Could you check a few things on this model? Use its own coordinates, in mm. A direction names the side the tool comes from. Coordinates: 2 decimals unless noted, no trailing zeros. Loops run counter-clockwise (first coordinate to the right, second up) from the corner with the lowest first, then second, coordinate; pieces in that order, holes last. Notation, with made-up numbers: (8, 69) - (18, 69) arc R15 ccw to (18, 79) - close; hole circle Ø4 at (-32.75, 65.25). An arc over 180 degrees is marked (long way). One line per question, with ' | ' between items. Start each with the question number.
1. I want a section at C-C, the plane x = 0. Write out the boundary of the cut face in (y, z).
2. I'm going to push flat-ended pins straight in: P1, Ø1.5, axis at x = -8, y = 4, coming from the -Z side; P2, Ø3, axis at y = 1, z = 1.5, coming from the -X side; P3, Ø2, axis at x = -4.5, y = 0.5, coming from the -Z side; P4, Ø1.8, axis at x = -10, y = 3, coming from the -Z side. Where does each tip first touch, or does it pass through?
3. We'd pull the mould along X, two halves only. Please class faces 1 (the cylindrical face through (12.5, 2.9, 0)), 2 (the cylindrical face through (8.8, 2.1, 0)), 3 (the flat face through (7, 3, 1.5)): pulls with the +X half, pulls with the -X half, needs draft (parallel to the pull), parting line crosses it, or undercut.
4. Which directions (+Z, -Z, +X, -X, +Y, -Y) give clear straight access to the entire face, cutting with the end or side of a thin tool? Please do faces 4 (the flat face through (-7, 3, -1.5)), 5 (the flat face through (7, 3, -1.5)), 6 (the flat face through (-7, 3, 1.5)).
5. I want a section at D-D, the plane y = 5.1. Write out the boundary of the cut face in (x, z), then the cut area to 3 significant figures.
6. I want a section at B-B, the plane y = 3. Write out the boundary of the cut face in (x, z), then the cut area to 3 significant figures.
7. Please list where these lines run through material, in increasing order: L1, parallel to Y at x = 10, z = 0.3; L2, parallel to Y at x = 6.75, z = 0; L3, parallel to Z at x = 5.5, y = 4.9. Write a range as [from, to].
8. I want a section at A-A, the plane z = 0. Write out the boundary of the cut face in (x, y), then the cut area to 3 significant figures.
from build123d import *

# Parameters (mm, degrees)
SKETCH1_R           = 4
SKETCH1_R_2         = 3
BOSS_EXTRUDE1_DEPTH = 6
SKETCH2_R           = 2.5
SKETCH2_R_2         = 1.5
BOSS_EXTRUDE2_DEPTH = 1.5


with BuildPart() as part:
    # Sketch1 → Boss-Extrude1 (new body)
    with BuildSketch(Plane(origin=(0, 0, 0), x_dir=(1, 0, 0), z_dir=(0, 1, 0))):
        with Locations(Location((0, 0, 0), (0, 0, 270))):
            Circle(SKETCH1_R)
        with Locations(Location((0, 0, 0), (0, 0, 270))):
            Circle(SKETCH1_R_2, mode=Mode.SUBTRACT)
    extrude(amount=BOSS_EXTRUDE1_DEPTH)

    # Sketch2 → Boss-Extrude2 (add, symmetric)
    # profile 1 of 4: a face of its own
    with BuildSketch(Plane.XY):
        with BuildLine():
            Line((-3, 5.5), (-10, 5.5))
            ThreePointArc((-10, 5.5), (-8.232233047, 4.767766953), (-7.5, 3))
            ThreePointArc((-7.5, 3), (-8.232233047, 1.232233047), (-10, 0.5))
            Line((-10, 0.5), (-3, 0.5))
            Line((-3, 0.5), (-3, 5.5))
        make_face()
    # profile 2 of 4: a face of its own
    with BuildSketch(Plane.XY):
        with Locations((-10, 3)):
            Circle(SKETCH2_R)
        with Locations((-10, 3)):
            Circle(SKETCH2_R_2, mode=Mode.SUBTRACT)
    # profile 3 of 4: a face of its own
    with BuildSketch(Plane.XY):
        with BuildLine():
            Line((3, 5.5), (3, 0.5))
            Line((3, 0.5), (10, 0.5))
            ThreePointArc((10, 0.5), (7.5, 3), (10, 5.5))
            Line((10, 5.5), (3, 5.5))
        make_face()
    # profile 4 of 4: a face of its own
    with BuildSketch(Plane.XY):
        with Locations((10, 3)):
            Circle(SKETCH2_R)
        with Locations((10, 3)):
            Circle(SKETCH2_R_2, mode=Mode.SUBTRACT)
    extrude(amount=BOSS_EXTRUDE2_DEPTH, both=True)


solid = part.part
Results are:
1) outline: (0, -4) - (6, -4) - (6, -3) - (0, -3) - close; (0, 3) - (6, 3) - (6, 4) - (0, 4) - close
2) P1: stops at z = -1.5 | P2: stops at x = -12.45 | P3: stops at z = -1.94 | P4: passes through
3) face 1: pulls with the +X half | face 2: undercut | face 3: needs draft
4) face 4: -Z, -X, +Y, -Y | face 5: -Z, +X, +Y, -Y | face 6: +Z, -X, +Y, -Y
5) outline: (-11.36, -1.5) - (-3.71, -1.5) arc R4 ccw to (3.71, -1.5) - (11.36, -1.5) - (11.36, 1.5) - (3.71, 1.5) arc R4 ccw to (-3.71, 1.5) - (-11.36, 1.5) - close; hole circle Ø6 at (0, 0) | area: 66.7 mm2
6) outline: (-12.5, -1.5) - (-11.5, -1.5) - (-11.5, 1.5) - (-12.5, 1.5) - close; (-8.5, -1.5) - (-3.71, -1.5) arc R4 ccw to (3.71, -1.5) - (8.5, -1.5) - (8.5, 1.5) - (3.71, 1.5) arc R4 ccw to (-3.71, 1.5) - (-8.5, 1.5) - close; (11.5, -1.5) - (12.5, -1.5) - (12.5, 1.5) - (11.5, 1.5) - close; hole circle Ø6 at (0, 0) | area: 55.6 mm2
7) L1: y = [0.5, 1.5], [4.5, 5.5] | L2: y = [0.5, 5.5] | L3: z = [-1.5, 1.5]
8) outline: (-10, 0.5) - (-4, 0.5) - (-4, 0) - (-3, 0) - (-3, 6) - (-4, 6) - (-4, 5.5) - (-10, 5.5) arc R2.5 ccw to start; (3, 0) - (4, 0) - (4, 0.5) - (10, 0.5) arc R2.5 ccw to (10, 5.5) - (4, 5.5) - (4, 6) - (3, 6) - close; hole circle Ø3 at (-10, 3); hole circle Ø3 at (10, 3) | area: 77.5 mm2
